```python
from build123d import *

# Parameters (mm, degrees)
SKETCH1_R           = 4
BOSS_EXTRUDE1_DEPTH = 10
SKETCH2_W           = 169.403995176
SKETCH2_H           = 40
BOSS_EXTRUDE2_DEPTH = 10
SKETCH3_W           = 10
SKETCH3_H           = 30
BOSS_EXTRUDE3_DEPTH = 80
SKETCH4_W           = 20
SKETCH4_H           = 5
BOSS_EXTRUDE4_DEPTH = 20
SKETCH5_R           = 4
CUT_EXTRUDE1_DEPTH  = 70
SKETCH6_R           = 6
CUT_EXTRUDE2_DEPTH  = 30


with BuildPart() as part:
    # Sketch1 → Boss-Extrude1 (new body)
    with BuildSketch(Plane.XY):
        with BuildLine():
            Line((-7.674547775, 2.258609406), (-16.579617078, -28))
            Line((-16.579617078, -28), (-22.35311977, -38))
            Line((-22.35311977, -38), (137.64688023, -38))
            Line((137.64688023, -38), (131.873377539, -28))
            Line((131.873377539, -28), (49.354955752, -28.3172709))
            Line((49.354955752, -28.3172709), (42, 0))
            ThreePointArc((42, 0), (34, 8), (26, 0))
            Line((26, 0), (18.4767103, -28))
            Line((18.4767103, -28), (13.916688293, -28))
            Line((13.916688293, -28), (7.674547775, 2.258609406))
            ThreePointArc((7.674547775, 2.258609406), (0, 8), (-7.674547775, 2.258609406))
        make_face()
        Circle(SKETCH1_R, mode=Mode.SUBTRACT)
        with Locations((34, 0)):
            Circle(SKETCH1_R, mode=Mode.SUBTRACT)
    extrude(amount=BOSS_EXTRUDE1_DEPTH)

    # Sketch2 → Boss-Extrude2 (add)
    with BuildSketch(Plane(origin=(0, -38, 0), x_dir=(-1, 0, 0), z_dir=(0, -1, 0))):
        with Locations((-61.414188083, -5)):
            Rectangle(SKETCH2_W, SKETCH2_H)
    extrude(amount=-BOSS_EXTRUDE2_DEPTH)

    # Sketch3 → Boss-Extrude3 (add)
    with BuildSketch(Plane(origin=(0, -28, 0), x_dir=(1, 0, 0), z_dir=(0, 1, 0))):
        with Locations((133.116185671, -5)):
            Rectangle(SKETCH3_W, SKETCH3_H)
    extrude(amount=BOSS_EXTRUDE3_DEPTH)

    # Sketch4 → Boss-Extrude4 (add)
    with BuildSketch(Plane.ZY.offset(-128.116185671)):
        with Locations((5, 46.5)):
            Rectangle(SKETCH4_W, SKETCH4_H)
        with Locations((5, -17.5)):
            Rectangle(SKETCH4_W, SKETCH4_H)
    extrude(amount=BOSS_EXTRUDE4_DEPTH)

    # Sketch5 → Cut-Extrude1 (cut)
    with BuildSketch(Plane(origin=(0, 49, 0), x_dir=(1, 0, 0), z_dir=(0, 1, 0))):
        with Locations(Location((115.116185671, -5, 0), (0, 0, 270))):
            Circle(SKETCH5_R)
        with BuildLine():
            Line((115.116185671, -15), (103.174329038, -18.113908317))
            Line((103.174329038, -18.113908317), (97.147243506, 5))
            Line((97.147243506, 5), (115.116185671, 5))
            ThreePointArc((115.116185671, 5), (105.116185671, -5), (115.116185671, -15))
        make_face()
    extrude(amount=-CUT_EXTRUDE1_DEPTH, mode=Mode.SUBTRACT)

    # Sketch6 → Cut-Extrude2 (cut)
    with BuildSketch(Plane(origin=(0, -28, 0), x_dir=(1, 0, 0), z_dir=(0, 1, 0))):
        with Locations(Location((115.116185671, -5, 0), (0, 0, 270))):
            Circle(SKETCH6_R)
    extrude(amount=-CUT_EXTRUDE2_DEPTH, mode=Mode.SUBTRACT)


solid = part.part
```
Geometry: final body of the model. Coordinates: model frame, mm. A direction names the side the tool comes from. Coordinates: 2 decimals unless noted, no trailing zeros. Order: outer loops, then holes, each group sorted by start corner. A loop starts at its lowest first (then second) coordinate and runs counter-clockwise, first axis right, second up. Notation, with made-up numbers: M 86,2.5 L 137,2.5 A10 ccw 137,19.5 Z; hole C -17.5,-37 d3. An arc over 180 degrees is marked long. Answer in a Markdown table with one row per item. Add a question column.
Q1. Section query D-D on x = 84. Return the cut outline in (y, z).
Q2. Section query C-C on z = 5. Count the separate pieces of the cut face and the enclosed holes in it, and give its area (3 significant figures).
Q3. Reachability of faces 1 (the cylindrical face through (111.29, 46.54, 14.24)), 2 (the flat face through (133, 11, -10)), 3 (the flat face through (133, 11, 20)), 4 (the flat face through (-2, -14, 0)) from +Z, -Z, +X, -X, +Y, -Y: full face, straight path, thin tool, end or side. Return the list, or none.
Q4. Line query: L1, parallel to X at y = 46.5, z = 5; L2, parallel to X at y = 2, z = 0.5; L3, parallel to X at y = -13, z = 6. Output: solid intervals per line, ascending.
Q5. Contact query for flat-ended pins moving along their axis: P1, Ø16, axis at x = 122, z = 4.5, coming from the +Y side; P2, Ø6.5, axis at x = 115.12, z = 5, coming from the -Y side; P3, Ø15.5, axis at x = 36.5, y = -12.5, coming from the +Z side; P4, Ø5.5, axis at y = -16.5, z = 3, coming from the -X side. Output: stop coordinate, or through.
Q6. Section query A-A on x = 0. Return the cut outline in (y, z).
Q7. Mould query, pull axis Y, two halves, no side actions, for faces 5 (the flat face through (122, -18, -5)), 6 (the flat face through (63, -38, 5)), 7 (the flat face through (10.84, -13.08, 4.93)), 8 (the flat face through (120, -15, 5)). Classes: released by +Y, released by -Y, zero draft, split by the parting line, or undercut.
Q8. Section query B-B on z = 18. Return the cut outline in (x, y).
Completed:
| question | item | result |
|---|---|---|
| 1 | outline | M -38,-15 L -28,-15 L -28,25 L -38,25 Z |
| 2 | separate pieces | 4 |
| 2 | enclosed holes | 2 |
| 2 | area | 3,910 mm2 |
| 3 | face 1 | +Z, -X, +Y |
| 3 | face 2 | -Z, +X, -X, +Y |
| 3 | face 3 | +Z, +X, -X, +Y |
| 3 | face 4 | -Z, -X, +Y |
| 4 | L1 | x = 108.12 to 111.12, 119.12 to 138.12 |
| 4 | L2 | x = -7.75 to -3.46, 3.46 to 7.73, 26.25 to 30.54, 37.46 to 41.75, 128.12 to 138.12 |
| 4 | L3 | x = -12.17 to 10.82, 22.51 to 45.38, 128.12 to 138.12 |
| 5 | P1 | stops at y = 52 |
| 5 | P2 | passes through |
| 5 | P3 | stops at z = 10 |
| 5 | P4 | stops at x = -14 |
| 6 | outline | M -38,-15 L -28,-15 L -28,0 L -4,0 L -4,10 L -28,10 L -28,25 L -38,25 Z; M 4,0 L 8,0 L 8,10 L 4,10 Z |
| 7 | face 5 | zero draft |
| 7 | face 6 | released by -Y |
| 7 | face 7 | released by +Y |
| 7 | face 8 | undercut |
| 8 | outline | M -23.29,-38 L 146.12,-38 L 146.12,-28 L 138.12,-28 L 138.12,52 L 128.12,52 L 128.12,-28 L -23.29,-28 Z |
